Job drawing, mm, ordinate dimensions from the low corner. One solid piece. A direction names the side the tool comes from. Round coordinates to 2 decimals unless told otherwise and drop trailing zeros. Write each loop counter-clockwise with the first axis right and the second up, starting at its lowest first coordinate (ties: lowest second). Pieces come first, ordered by that corner, then holes. Notation, with made-up numbers: (81, -30.5) -> (85, -30.5) arc R17 ccw to (85, -16.5) -> close; hole circle Ø1 at (59, 23). An arc over 180 degrees is marked (long way). Use CSV: the item, a comma, the result in double quotes. Start each with the question number.
(1) Saw through at B-B (x = 55). Give the cut face in (y, z).
(2) Saw through at A-A (x = 20). Give the cut face in (y, z), plus the area to 3 significant figures.
(3) Two-plate mould, pull along Z, no slides. Class the marked faces 1, 2 and 3: released by +Z, released by -Z, zero draft, split by the parting line, or undercut.
(4) Probe line 1 (X direction, y = 33.3, z = 20); line 2 (Z direction, x = 55, y = 6.5); line 3 (X direction, y = 39, z = 69). List the from-to ranges inside material, lowest first. Write a range as [from, to].
(5) Drop flat-ended pins along their axis: pin 1 (25 mm diameter, centred on x = 65.5, z = 29, fed in from +Y); pin 2 (13 mm diameter, centred on x = 104.5, z = 53, fed in from +Y); pin 3 (3 mm diameter, centred on x = 71.5, y = 38.5, fed in from -Z); pin 4 (11 mm diameter, centred on y = 14, z = 96, fed in from +X). Give the stop position or say it passes through.
(6) Which spindle directions (+Z, -Z, +X, -X, +Y, -Y) get a long thin tool onto all of the face, cutting with end or side? Do the marked faces 4, 5, 6, 7 and 8. Say none if no direction does.
(7) Saw through at D-D (y = 65). Give the cut face in (x, z).
(8) Saw through at C-C (y = 23). Give the cut face in (x, z).
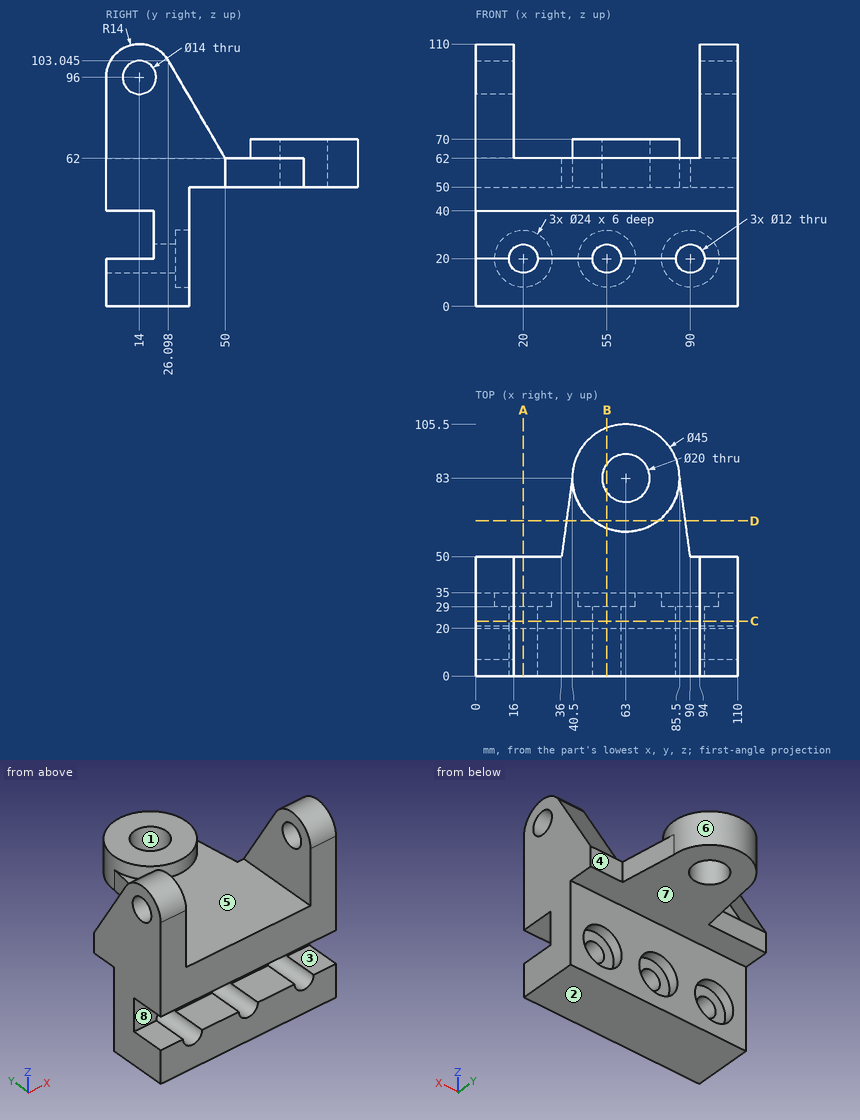
Answers:
1,outline,"(0, 0) -> (35, 0) -> (35, 8) -> (29, 8) -> (29, 14) -> (0, 14) -> close; (0, 40) -> (20, 40) -> (20, 26) -> (29, 26) -> (29, 32) -> (35, 32) -> (35, 50) -> (77, 50) -> (77, 70) -> (61.97, 70) -> (61.97, 62) -> (0, 62) -> close; (89, 50) -> (104.03, 50) -> (104.03, 70) -> (89, 70) -> close"
2,outline,"(0, 0) -> (35, 0) -> (35, 8) -> (29, 8) -> (29, 14) -> (0, 14) -> close; (0, 40) -> (20, 40) -> (20, 26) -> (29, 26) -> (29, 32) -> (35, 32) -> (35, 50) -> (50, 50) -> (50, 62) -> (0, 62) -> close"
2,area,"1,580 mm²"
3,face 1,"zero draft"
3,face 2,"released by -Z"
3,face 3,"undercut"
4,line 1,"x = [0, 8], [32, 43], [67, 78], [102, 110]"
4,line 2,"z = [0, 14], [40, 62]"
4,line 3,"x = [0, 16], [94, 110]"
5,pin 1,"stops at y = 35"
5,pin 2,"stops at y = 50"
5,pin 3,"stops at z = 50"
5,pin 4,"passes through"
6,face 4,"+Z, -Z, +X, +Y"
6,face 5,"+Z, -Y"
6,face 6,"+Z"
6,face 7,"-Z, +X, -X, +Y"
6,face 8,"+X, -X, -Y"
7,outline,"(38.05, 50) -> (87.95, 50) -> (87.95, 62) -> (76.5, 62) -> (76.5, 70) -> (49.5, 70) -> (49.5, 62) -> (38.05, 62) -> close"
8,outline,"(0, 0) -> (110, 0) -> (110, 106.72) -> (94, 106.72) -> (94, 62) -> (16, 62) -> (16, 106.72) -> (0, 106.72) -> close; hole circle Ø12 at (20, 20); hole circle Ø12 at (55, 20); hole circle Ø12 at (90, 20)"
